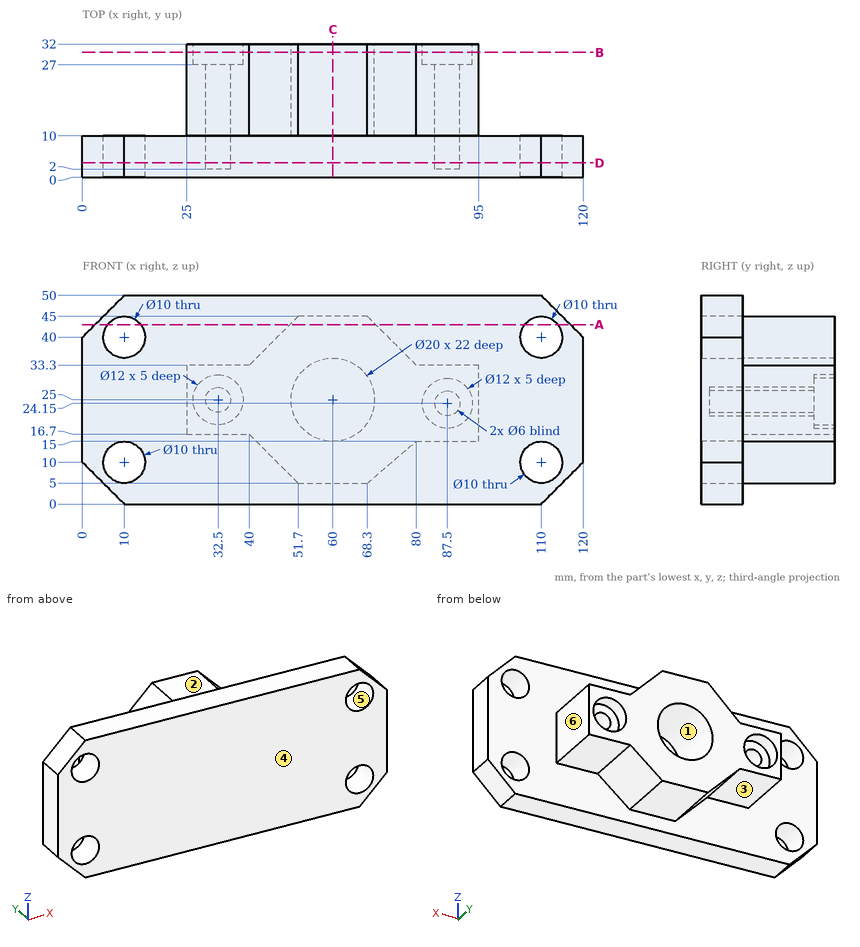
Answer from the drawing. Dimensions are ordinates in mm from the lowest x, y and z of the part. A direction names the side the tool comes from. Coordinates: 2 decimals unless noted, no trailing zeros. Order: outer loops, then holes, each group sorted by start corner. A loop starts at its lowest first (then second) coordinate and runs counter-clockwise, first axis right, second up. Notation, with made-up numbers: (6, -39.5) -> (35, -39.5) arc R37 ccw to (35, -2.5) -> close; hole circle Ø3 at (64.5, 52). An arc over 180 degrees is marked (long way). Answer as a JSON object with one key per item and string values.
1) A cutting plane is placed at D-D, the plane y = 3.5. Determine the outline of the cut face in (x, z).
Model answer:
{"outline": "(0, 10) -> (10, 0) -> (110, 0) -> (120, 10) -> (120, 40) -> (110, 50) -> (10, 50) -> (0, 40) -> close; hole circle Ø10 at (10, 10); hole circle Ø10 at (10, 40); hole circle Ø6 at (32.5, 25); hole circle Ø6 at (87.5, 24.15); hole circle Ø10 at (110, 10); hole circle Ø10 at (110, 40)"}
2) A tool of negligible diameter and unlimited length cuts with its end or side. For the marked faces 1, 2 and 3, from which of +Z, -Z, +X, -X, +Y, -Y can it reach the whole face along a straight path? Write none if from no direction.
Model answer:
{"face 1": "+Y", "face 2": "+Z, +X, -X, +Y", "face 3": "-Z, -X, +Y"}
3) Each of these flat-tipped pins is pushed along its axis until it touches: pin 1 (3.5 mm diameter, centred on x = 85, z = 23.5, fed in from +Y); pin 2 (1 mm diameter, centred on y = 8, z = 42, fed in from -X); pin 3 (7.5 mm diameter, centred on x = 31, y = 17, fed in from +Z). Where does it stop, or does it pass through?
Model answer:
{"pin 1": "stops at y = 27", "pin 2": "stops at x = 1.5", "pin 3": "stops at z = 33.3"}
4) A cutting plane is placed at C-C, the plane x = 60. Determine the outline of the cut face in (y, z), plus the area to 3 significant figures.
Model answer:
{"outline": "(0, 0) -> (10, 0) -> (10, 5) -> (32, 5) -> (32, 15) -> (10, 15) -> (10, 35) -> (32, 35) -> (32, 45) -> (10, 45) -> (10, 50) -> (0, 50) -> close", "area": "940 mm²"}
5) A cutting plane is placed at A-A, the plane z = 43. Determine the outline of the cut face in (x, y), plus the area to 3 significant figures.
Model answer:
{"outline": "(3, 0) -> (6, 0) -> (6, 10) -> (3, 10) -> close; (14, 0) -> (106, 0) -> (106, 10) -> (70.3, 10) -> (70.3, 32) -> (49.7, 32) -> (49.7, 10) -> (14, 10) -> close; (114, 0) -> (117, 0) -> (117, 10) -> (114, 10) -> close", "area": "1,430 mm²"}
6) A cutting plane is placed at B-B, the plane y = 30. Determine the outline of the cut face in (x, z), plus the area to 3 significant figures.
Model answer:
{"outline": "(25, 16.7) -> (40, 16.7) -> (51.7, 5) -> (68.3, 5) -> (80, 15) -> (95, 15) -> (95, 33.3) -> (80, 33.3) -> (68.3, 45) -> (51.7, 45) -> (40, 33.3) -> (25, 33.3) -> close; hole circle Ø12 at (32.5, 25); hole circle Ø20 at (60, 25); hole circle Ø12 at (87.5, 24.15)", "area": "1,320 mm²"}
7) The mould has two halves that part along X. Classify the marked faces 4, 5 and 6: released by +X, released by -X, zero draft, split by the parting line, or undercut.
Model answer:
{"face 4": "zero draft", "face 5": "undercut", "face 6": "released by +X"}
8) Consider line 1 along X through (y, z) = (5, 40); line 2 along X through (y, z) = (21, 24); line 3 along X through (y, z) = (13, 25). Determine where each line is inside the solid, lowest interval first. Write a range as from..to.
Model answer:
{"line 1": "x = 0..5, 15..105, 115..120", "line 2": "x = 25..29.67, 35.33..50.05, 69.95..84.5, 90.5..95", "line 3": "x = 25..29.5, 35.5..50, 70..84.62, 90.38..95"}
